from build123d import *

# Parameters (mm, degrees)
SKETCH1_R           = 40
SKETCH1_R_2         = 31.75
BOSS_EXTRUDE1_DEPTH = 3
SKETCH3_R           = 1.75
CUT_EXTRUDE2_DEPTH  = 57.648036153
CIRPATTERN1_COUNT   = 6
SKETCH5_R           = 3.25
CUT_EXTRUDE4_DEPTH  = 1
CIRPATTERN2_COUNT   = 6
SKETCH6_W           = 3.5
SKETCH6_H           = 6.5
CUT_EXTRUDE5_DEPTH  = 1
CIRPATTERN3_COUNT   = 6


with BuildPart() as part:
    # Sketch1 → Boss-Extrude1 (new body)
    with BuildSketch(Plane(origin=(0, 0, 0), x_dir=(1, 0, 0), z_dir=(0, 1, 0))):
        with Locations(Location((0, 0, 0), (0, 0, 270))):
            Circle(SKETCH1_R)
        with Locations(Location((0, 0, 0), (0, 0, 270))):
            Circle(SKETCH1_R_2, mode=Mode.SUBTRACT)
    extrude(amount=BOSS_EXTRUDE1_DEPTH)

    # Sketch3 → Cut-Extrude2 (cut, through all)
    with BuildSketch(Plane.XZ):
        with Locations(Location((37, 0, 0), (0, 0, 270))):
            Circle(SKETCH3_R)
    cut_extrude2 = extrude(amount=-CUT_EXTRUDE2_DEPTH, mode=Mode.SUBTRACT)

    # CirPattern1: Cut-Extrude2 ×6 about axis
    cirpattern1_axis = Axis((0, 0, 0), (0, 1, 0))
    for i in range(1, CIRPATTERN1_COUNT):
        add(cut_extrude2.rotate(cirpattern1_axis, i * 360 / CIRPATTERN1_COUNT), mode=Mode.SUBTRACT)

    # Sketch5 → Cut-Extrude4 (cut)
    with BuildSketch(Plane.XZ):
        with Locations((18.5, 32.04293994)):
            Circle(SKETCH5_R)
    cut_extrude4 = extrude(amount=-CUT_EXTRUDE4_DEPTH, mode=Mode.SUBTRACT)

    # CirPattern2: Cut-Extrude4 ×6 about axis
    cirpattern2_axis = Axis((0, 0, 0), (0, 1, 0))
    for i in range(1, CIRPATTERN2_COUNT):
        add(cut_extrude4.rotate(cirpattern2_axis, i * 360 / CIRPATTERN2_COUNT), mode=Mode.SUBTRACT)

    # Sketch6 → Cut-Extrude5 (cut)
    with BuildSketch(Plane.XZ):
        with Locations((38.75, 0)):
            Rectangle(SKETCH6_W, SKETCH6_H)
    cut_extrude5 = extrude(amount=-CUT_EXTRUDE5_DEPTH, mode=Mode.SUBTRACT)

    # CirPattern3: Cut-Extrude5 ×6 about axis
    cirpattern3_axis = Axis((0, 0, 0), (0, 1, 0))
    for i in range(1, CIRPATTERN3_COUNT):
        add(cut_extrude5.rotate(cirpattern3_axis, i * 360 / CIRPATTERN3_COUNT), mode=Mode.SUBTRACT)


solid = part.part
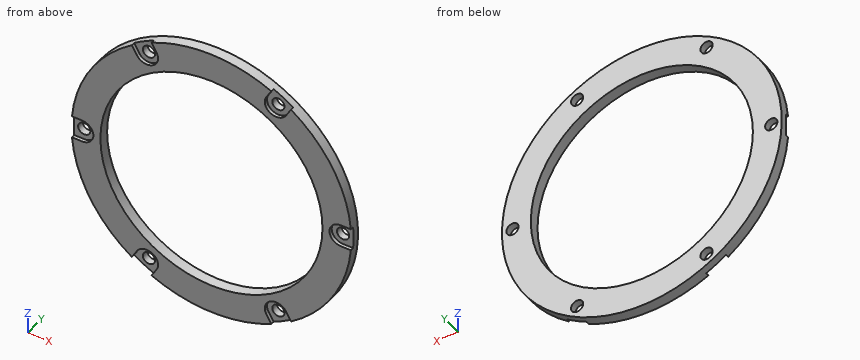
The listing builds one solid part. Answer for the finished solid, in the listing's coordinates (mm). Round coordinates to 2 decimals unless told otherwise and drop trailing zeros. Order: outer loops, then holes, each group sorted by start corner. A loop starts at its lowest first (then second) coordinate and runs counter-clockwise, first axis right, second up. Notation, with made-up numbers: (-40, 37) -> (-11, 37) arc R29 ccw to (-11, 74) -> close; hole circle Ø2 at (77, 3). An arc over 180 degrees is marked (long way). Put each result on its own line as item: value.
Q1. Section B-B, the plane z = -23.5 is taken. Write down the section's boundary in (x, y).
Results list:
outline: (-32.37, 0) -> (-21.35, 0) -> (-21.35, 3) -> (-32.37, 3) -> close; (21.35, 0) -> (32.37, 0) -> (32.37, 3) -> (21.35, 3) -> close
Q2. Section C-C, the plane y = 1.75 is taken. Write down the section's boundary in (x, z).
Results list:
outline: circle Ø80 at (0, 0); hole circle Ø3.5 at (-37, 0); hole circle Ø63.5 at (0, 0); hole circle Ø3.5 at (-18.5, -32.04); hole circle Ø3.5 at (-18.5, 32.04); hole circle Ø3.5 at (18.5, -32.04); hole circle Ø3.5 at (18.5, 32.04); hole circle Ø3.5 at (37, 0)
Q3. Consider line 1 along X through (y, z) = (2.45, 0); line 2 along X through (y, z) = (2.55, -24.5); line 3 along Z through (x, y) = (-10, 1.05). Determine where each line is inside the solid, lowest interval first.
Results list:
line 1: -40 to -38.75, -35.25 to -31.75, 31.75 to 35.25, 38.75 to 40
line 2: -31.62 to -20.19, 20.19 to 31.62
line 3: -38.73 to -30.13, 30.13 to 38.73
Q4. Section A-A, the plane x = 0 is taken. Write down the section's boundary in (y, z), and give its area (3 significant figures).
Results list:
outline: (0, -40) -> (3, -40) -> (3, -31.75) -> (0, -31.75) -> close; (0, 31.75) -> (3, 31.75) -> (3, 40) -> (0, 40) -> close
area: 49.5 mm^2
Q5. Section D-D, the plane x = -19 is taken. Write down the section's boundary in (y, z).
Results list:
outline: (0, -28.83) -> (1, -28.83) -> (1, -30.37) -> (3, -30.37) -> (3, -25.44) -> (0, -25.44) -> close; (0, 25.44) -> (3, 25.44) -> (3, 30.37) -> (1, 30.37) -> (1, 28.83) -> (0, 28.83) -> close; (1, -35.2) -> (3, -35.2) -> (3, -33.72) -> (1, -33.72) -> close; (1, 33.72) -> (3, 33.72) -> (3, 35.2) -> (1, 35.2) -> close
Q6. Each of these flat-tipped pins is pushed along its axis until it touches: P1, Ø5, axis at x = 30, z = 6.5, coming from the +Y side; P2, Ø1.9, axis at x = 36.5, z = 1, coming from the -Y side. Where does it stop, or does it pass through?
Results list:
P1: y = 3
P2: y = 1
